Can you work these out from the model? Positions are in its coordinate system, mm. A direction names the side the tool comes from. Coordinates: 2 decimals unless noted, no trailing zeros. Write each loop counter-clockwise with the first axis right and the second up, starting at its lowest first coordinate (ties: lowest second). Pieces come first, ordered by that corner, then holes. Notation, with made-up numbers: M -2,37 L 14,37 A22 ccw 14,44 Z; hole C 85,68.25 d7. An arc over 180 degrees is marked long. Use one line per item in the form item = value. Start each with the question number.
```python
from build123d import *

# Parameters (mm, degrees)
HOUSING_BLOCK_SKETCH_W = 116
HOUSING_BLOCK_SKETCH_H = 70
HOUSING_BLOCK_DEPTH    = 96
MOUNTING_FLANGE_DEPTH  = 12
FLANGE_PAD_DEPTH       = 3
FLANGE_HOLE_SKETCH_R   = 10
FLANGE_HOLE_DEPTH      = 198.002538055
TOP_BOSS_SKETCH_R      = 23
TOP_BOSS_SKETCH_R_2    = 12
TOP_BOSS_46_DEPTH      = 25
GUSSET_DEPTH           = 10


with BuildPart() as part:
    # Housing Block Sketch → Housing Block (new body)
    with BuildSketch(Plane.XY):
        with Locations((58, 35)):
            Rectangle(HOUSING_BLOCK_SKETCH_W, HOUSING_BLOCK_SKETCH_H)
    extrude(amount=HOUSING_BLOCK_DEPTH)

    # Mounting Flange Sketch → Mounting Flange (add)
    with BuildSketch(Plane(origin=(0, 0, 0), x_dir=(1, 0, 0), z_dir=(0, 1, 0))):
        with BuildLine():
            Line((116, 0), (116, -96))
            Line((116, -96), (153.08596721, -67.935234971))
            ThreePointArc((153.08596721, -67.935234971), (163, -48), (153.08596721, -28.064765029))
            Line((153.08596721, -28.064765029), (116, 0))
        make_face()
    mounting_flange = extrude(amount=MOUNTING_FLANGE_DEPTH)

    # Flange Pad Sketch → Flange Pad (add)
    with BuildSketch(Plane(origin=(0, 12, 0), x_dir=(1, 0, 0), z_dir=(0, 1, 0))):
        with BuildLine():
            Line((138, -28), (116, -28))
            Line((116, -28), (116, -68))
            Line((116, -68), (138, -68))
            ThreePointArc((138, -68), (158, -48), (138, -28))
        make_face()
    flange_pad = extrude(amount=FLANGE_PAD_DEPTH)

    # Flange Hole Sketch → Flange Hole (cut, through all)
    with BuildSketch(Plane(origin=(0, 15, 0), x_dir=(1, 0, 0), z_dir=(0, 1, 0))):
        with Locations(Location((138, -48, 0), (0, 0, 270))):
            Circle(FLANGE_HOLE_SKETCH_R)
    flange_hole = extrude(amount=-FLANGE_HOLE_DEPTH, mode=Mode.SUBTRACT)

    # Flange Mirror: Mounting Flange, Flange Pad, Flange Hole across plane
    add(mounting_flange.mirror(Plane(origin=(58, 0, 0), x_dir=(0, 0, 1), z_dir=(1, 0, 0))))
    add(flange_pad.mirror(Plane(origin=(58, 0, 0), x_dir=(0, 0, 1), z_dir=(1, 0, 0))))
    add(flange_hole.mirror(Plane(origin=(58, 0, 0), x_dir=(0, 0, 1), z_dir=(1, 0, 0))), mode=Mode.SUBTRACT)

    # Top Boss Sketch → Top Boss Ø46 (add)
    with BuildSketch(Plane(origin=(0, 70, 0), x_dir=(1, 0, 0), z_dir=(0, 1, 0))):
        with Locations(Location((58, -48, 0), (0, 0, 90))):
            Circle(TOP_BOSS_SKETCH_R)
        with Locations(Location((58, -48, 0), (0, 0, 270))):
            Circle(TOP_BOSS_SKETCH_R_2, mode=Mode.SUBTRACT)
    extrude(amount=TOP_BOSS_46_DEPTH)

    # Gusset Sketch → Gusset (add, symmetric)
    with BuildSketch(Plane.XY.offset(47.5)):
        Polygon((81, 70), (116, 70), (72.155995343, 95), (72.155995343, 70), align=None)
    gusset = extrude(amount=GUSSET_DEPTH, both=True)

    # Gusset Mirror: Gusset across plane
    add(gusset.mirror(Plane(origin=(58, 0, 0), x_dir=(0, 0, 1), z_dir=(1, 0, 0))))


solid = part.part
```
1) Suppose I cut it at C-C on x = 58. Please give me the cut outline in (y, z), and give its area (3 significant figures).
2) Which directions (+Z, -Z, +X, -X, +Y, -Y) give clear straight access to the entire face, cutting with the end or side of a thin tool? Please do faces 1 (the face through (27, 76, 57.5)), 2 (the face through (158, 13, 48)), 3 (the face through (89, 76, 37.5)).
3) Please list where these lines run through material, in increasing order: line 1 (X direction, y = 8, z = 48); line 2 (X direction, y = 20, z = 92); line 3 (X direction, y = 86.5, z = 52).
4) Suppose I cut it at A-A on x = 142.5. Please give me the cut outline in (y, z), and give its area (3 significant figures).
5) If we mould it in two halves opening along X, with no side actions, what happens to faces 4 (the face through (46.285, 82.325, 45.399)), 5 (the face through (134.803, 5.916, 14.229)), 6 (the face through (57, 35, 96))? For each: +X half, -X half, draft (parallel to the pull), parting line (faces both ways), or undercut.
6) Suppose I cut it at D-D on y = 51. Please give me the cut outline in (x, z), and give its area (3 significant figures).
7) Suppose I cut it at B-B on z = 48. Please give me the cut outline in (x, y).
8) Will these pins go through, and if not, where does the flat tip stop? pin 1 Ø0.9 at (x, y) = (130, 13.5) entering from -Z; pin 2 Ø18 at (x, z) = (138, 48) entering from -Y; pin 3 Ø6 at (y, z) = (67.5, 26.5) entering from -X; pin 4 Ø23.5 at (x, z) = (144.5, 71.5) entering from +Y.
Computed values:
q1.outline = M 0,0 L 70,0 L 70,25 L 95,25 L 95,36 L 70,36 L 70,60 L 95,60 L 95,71 L 70,71 L 70,96 L 0,96 Z
q1.area = 7,270 mm²
q2.face_1 = +Z, -X, +Y
q2.face_2 = +X, +Y
q2.face_3 = -Z, +X, +Y
q3.line_1 = -47 to -32, -12 to 128, 148 to 163
q3.line_2 = 0 to 116
q3.line_3 = 28.94 to 46.69, 69.31 to 87.06
q4.outline = M 0,20.05 L 12,20.05 L 12,28.51 L 15,28.51 L 15,39.07 L 0,39.07 Z; M 0,56.93 L 15,56.93 L 15,67.49 L 12,67.49 L 12,75.95 L 0,75.95 Z
q4.area = 520 mm²
q5.face_4 = undercut
q5.face_5 = +X half
q5.face_6 = draft
q6.outline = M 0,0 L 116,0 L 116,96 L 0,96 Z
q6.area = 11,100 mm²
q7.outline = M -47,0 L -32,0 L -32,15 L -42,15 L -42,12 L -47,12 Z; M -12,0 L 128,0 L 128,15 L 116,15 L 116,70 L 81,89.96 L 81,95 L 70,95 L 70,70 L 46,70 L 46,95 L 35,95 L 35,89.96 L 0,70 L 0,15 L -12,15 Z; M 148,0 L 163,0 L 163,12 L 158,12 L 158,15 L 148,15 Z
q8.pin_1 = 28
q8.pin_2 = through
q8.pin_3 = 0
q8.pin_4 = 15
